```python
from build123d import *

# Parameters (mm, degrees)
SKETCH_1_W          = 320
SKETCH_1_H          = 140
EXTRUDE_1_DEPTH     = 6
SKETCH_2_R          = 4.5
CUT_EXTRUDE_1_DEPTH = 16


with BuildPart() as part:
    # 草图1 → 凸台-拉伸1 (new, symmetric)
    with BuildSketch(Plane.XY):
        Rectangle(SKETCH_1_W, SKETCH_1_H)
    extrude(amount=EXTRUDE_1_DEPTH, both=True)

    # 草图2 → 切除-拉伸1 (cut, symmetric)
    with BuildSketch(Plane.XY):
        with Locations((-125, -40)):
            Circle(SKETCH_2_R)
        with Locations((125, 40)):
            Circle(SKETCH_2_R)
    extrude(amount=CUT_EXTRUDE_1_DEPTH, both=True, mode=Mode.SUBTRACT)


solid = part.part
```
Geometry check sheet. Reference: the model listing, model coordinates, mm. Give positions to 0.01 mm unless a question says otherwise; leave off trailing zeros. Write each loop counter-clockwise with the first axis right and the second up, starting at its lowest first coordinate (ties: lowest second). Pieces come first, ordered by that corner, then holes. Notation, with made-up numbers: (-11, 29) - (29, 29) arc R20 cw to (29, 50) - close; hole circle Ø9 at (59.25, -5.5). An arc over 180 degrees is marked (long way). Use a Markdown table: item, result.
Q1. Section check A-A, the plane y = -40. Enter the section's corners in (x, z).
Computed:
| item | result |
|---|---|
| outline | (-160, -6) - (-129.5, -6) - (-129.5, 6) - (-160, 6) - close; (-120.5, -6) - (160, -6) - (160, 6) - (-120.5, 6) - close |
Q2. Section check B-B, the plane x = -125. Enter the section's corners in (y, z).
Computed:
| item | result |
|---|---|
| outline | (-70, -6) - (-44.5, -6) - (-44.5, 6) - (-70, 6) - close; (-35.5, -6) - (70, -6) - (70, 6) - (-35.5, 6) - close |
Q3. Draft check along Y on faces 1 (the face through (-2, -70, 0)), 2 (the face through (-128.6, -42.7, 0.1)), 3 (the face through (-2, 70, 0)), 4 (the face through (-2, 1, 6)). Enter one of: pulls with the +Y half, pulls with the -Y half, needs draft (parallel to the pull), parting line crosses it, or undercut.
Computed:
| item | result |
|---|---|
| face 1 | pulls with the -Y half |
| face 2 | undercut |
| face 3 | pulls with the +Y half |
| face 4 | needs draft |
Q4. Thickness scan on L1, parallel to X at y = -40, z = -2.25; L2, parallel to Y at x = -125, z = 0; L3, parallel to Y at x = 125, z = -3.5. Record the ranges inside material, lowest first. Write a range as [from, to].
Computed:
| item | result |
|---|---|
| L1 | x = [-160, -129.5], [-120.5, 160] |
| L2 | y = [-70, -44.5], [-35.5, 70] |
| L3 | y = [-70, 35.5], [44.5, 70] |
